Geometry: see drawing. Coordinates: mm, zero at the bounding-box minimum. Round coordinates to 2 decimals unless told otherwise and drop trailing zeros. Write each loop counter-clockwise with the first axis right and the second up, starting at its lowest first coordinate (ties: lowest second). Pieces come first, ordered by that corner, then holes.
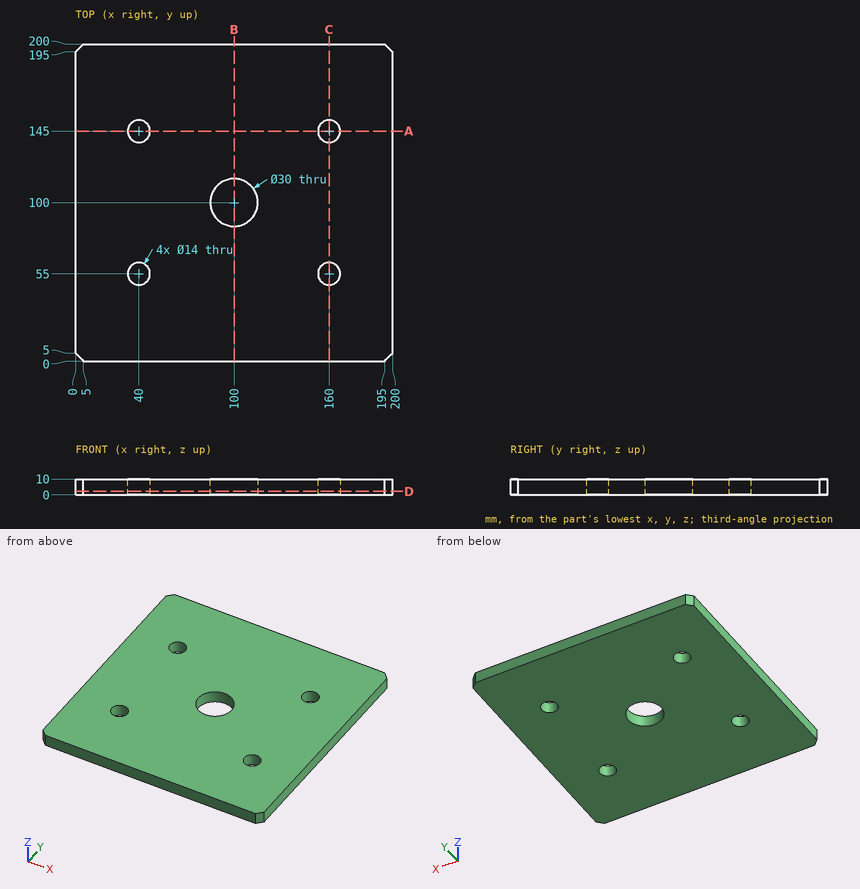
1) Section query A-A on y = 145. Return the cut outline in (x, z), then the cut area to 3 significant figures.
Taken from the geometry:
outline: (0, 0) - (33, 0) - (33, 10) - (0, 10) - close; (47, 0) - (153, 0) - (153, 10) - (47, 10) - close; (167, 0) - (200, 0) - (200, 10) - (167, 10) - close
area: 1,720 mm2
2) Material intervals for line 1 (Y direction, x = 160, z = 5.75); line 2 (Y direction, x = 100, z = 6.5); line 3 (Y direction, x = 163, z = 6), sorted ascending.
Taken from the geometry:
line 1: y = 0 to 48, 62 to 138, 152 to 200
line 2: y = 0 to 85, 115 to 200
line 3: y = 0 to 48.68, 61.32 to 138.68, 151.32 to 200
3) Section query B-B on x = 100. Return the cut outline in (y, z), then the cut area to 3 significant figures.
Taken from the geometry:
outline: (0, 0) - (85, 0) - (85, 10) - (0, 10) - close; (115, 0) - (200, 0) - (200, 10) - (115, 10) - close
area: 1,700 mm2
4) Section query D-D on z = 2.25. Return the cut outline in (x, y), then the cut area to 3 significant figures.
Taken from the geometry:
outline: (0, 5) - (5, 0) - (195, 0) - (200, 5) - (200, 195) - (195, 200) - (5, 200) - (0, 195) - close; hole circle Ø14 at (40, 55); hole circle Ø14 at (40, 145); hole circle Ø30 at (100, 100); hole circle Ø14 at (160, 55); hole circle Ø14 at (160, 145)
area: 38,600 mm2
5) Section query C-C on x = 160. Return the cut outline in (y, z).
Taken from the geometry:
outline: (0, 0) - (48, 0) - (48, 10) - (0, 10) - close; (62, 0) - (138, 0) - (138, 10) - (62, 10) - close; (152, 0) - (200, 0) - (200, 10) - (152, 10) - close
6) Contact query for a flat-ended pin moving along its axis: P1, Ø24, axis at x = 100, y = 100, coming from the +Z side. Output: stop coordinate, or through.
Taken from the geometry:
P1: passes through
